```python
from build123d import *

# Parameters (mm, degrees)
UPRIGHT_V_NOTCH_PLATE_DEPTH = 12
BASE_PLATE_SKETCH_W         = 80
BASE_PLATE_SKETCH_H         = 15
BASE_PLATE_DEPTH            = 40
BASE_HOLE_SKETCH_24_R       = 12
BASE_HOLE_24_DEPTH          = 20


with BuildPart() as part:
    # Upright V-Notch Profile Sketch → Upright V-Notch Plate (new body)
    with BuildSketch(Plane.XY):
        Polygon((0, 0), (0, -50), (80, -50), (80, 0), (60, 0), (50, -16), (30, -16), (20, 0), align=None)
    extrude(amount=UPRIGHT_V_NOTCH_PLATE_DEPTH)

    # Base Plate Sketch → Base Plate (add)
    with BuildSketch(Plane.XY.offset(12)):
        with Locations((40, -42.5)):
            Rectangle(BASE_PLATE_SKETCH_W, BASE_PLATE_SKETCH_H)
    extrude(amount=BASE_PLATE_DEPTH)

    # Base Hole Sketch Ø24 → Base Hole Ø24 (cut)
    with BuildSketch(Plane(origin=(0, -35, 0), x_dir=(1, 0, 0), z_dir=(0, 1, 0))):
        with Locations(Location((40, -32, 0), (0, 0, 270))):
            Circle(BASE_HOLE_SKETCH_24_R)
    extrude(amount=-BASE_HOLE_24_DEPTH, mode=Mode.SUBTRACT)


solid = part.part
```
For this review, take the finished solid that the model builds, in its own axes (mm). A direction names the side the tool comes from. Give positions to 0.01 mm unless a question says otherwise; leave off trailing zeros. Write each loop counter-clockwise with the first axis right and the second up, starting at its lowest first coordinate (ties: lowest second). Pieces come first, ordered by that corner, then holes. Notation, with made-up numbers: M 17.25,41.25 L 32.25,41.25 A20 ccw 32.25,52.25 Z; hole C 83.25,-10 d6. An arc over 180 degrees is marked long. Answer as a JSON object with one key per item and string values. Group by question number.
Item 1: Consider section D-D on y = -9.5. Write out the cut boundary in (x, z), plus the area to 4 significant figures.
Item 2: Tool access review of faces 1 (the flat face through (10, 0, 6)), 2 (the flat face through (31, -35, 23)), 3 (the flat face through (40, -16, 6)): name each direction out of +Z, -Z, +X, -X, +Y, -Y from which nothing blocks a thin tool from reaching the whole face with its end or side.
Item 3: For probe 1 along X at (y, z) = (-42, 32); probe 2 along Y at (x, z) = (10, 37); probe 3 along Z at (x, y) = (52, -16), list the stretches that pass through material, from the lowest coordinate up. Write a range as [from, to].
Item 4: Consider section A-A on z = 32. Write out the cut boundary in (x, y).
Item 5: For pin 1 Ø4 at (x, y) = (71, -12.5) entering from +Z; pin 2 Ø9.5 at (x, z) = (45, 9) entering from +Y, all flat-tipped, find the tip position at first contact; note any pin that passes through.
Item 6: Draft analysis for pull direction Z (two halves, no side actions). For faces 4 (the flat face through (55, -8, 6)), 5 (the flat face through (39, -25, 0)), 6 (the flat face through (39, -21, 12)), 7 (the cylindrical face through (35.404, -42.395, 43.085)), state which applies: +Z half, -Z half, draft (parallel to the pull), parting line (faces both ways), or undercut.
Item 7: Consider section B-B on x = 40. Write out the cut boundary in (y, z).
Item 8: Consider section C-C on z = 5.5. Write out the cut boundary in (x, y), plus the area to 3 significant figures.
Check result:
{
 "1": {"outline": "M 0,0 L 25.94,0 L 25.94,12 L 0,12 Z; M 54.06,0 L 80,0 L 80,12 L 54.06,12 Z", "area": "622.5 mm^2"},
 "2": {"face 1": "+Z, -Z, +X, -X, +Y", "face 2": "+Z, +X, -X, +Y", "face 3": "+Z, -Z, +Y"},
 "3": {"probe 1": "x = [0, 28], [52, 80]", "probe 2": "y = [-50, -35]", "probe 3": "z = [0, 12]"},
 "4": {"outline": "M 0,-50 L 28,-50 L 28,-35 L 0,-35 Z; M 52,-50 L 80,-50 L 80,-35 L 52,-35 Z"},
 "5": {"pin 1": "stops at z = 12", "pin 2": "stops at y = -16"},
 "6": {"face 4": "draft", "face 5": "-Z half", "face 6": "+Z half", "face 7": "undercut"},
 "7": {"outline": "M -50,0 L -16,0 L -16,12 L -35,12 L -35,20 L -50,20 Z; M -50,44 L -35,44 L -35,52 L -50,52 Z"},
 "8": {"outline": "M 0,-50 L 80,-50 L 80,0 L 60,0 L 50,-16 L 30,-16 L 20,0 L 0,0 Z", "area": "3,520 mm^2"}
}
